Source: CAD feature listing. Evaluate the final solid. Frame: model axes, mm. A direction names the side the tool comes from. Round coordinates to 2 decimals unless told otherwise and drop trailing zeros. Order: outer loops, then holes, each group sorted by start corner. A loop starts at its lowest first (then second) coordinate and runs counter-clockwise, first axis right, second up. Notation, with made-up numbers: (66.5, -27) - (108.5, -27) arc R27 ccw to (108.5, 5) - close; hole circle Ø5 at (72, -30.75). An arc over 180 degrees is marked (long way). Put each result on its own line as item: value. Start each with the question number.
1) Contact query for a flat-ended pin moving along its axis: P1, Ø10.5, axis at x = 305, z = -50, coming from the -Y side. Output: stop coordinate, or through.
2) Section B-B on y = 7.25. State how many separate pieces and enclosed holes the cut face has, then the cut area to 3 significant figures.
3) Access query for faces 5 (the face through (320, 10, 1)), 6 (the face through (-150, 10, 220)), 7 (the face through (-320, 10, -1)). Directions: +Z, -Z, +X, -X, +Y, -Y. A direction counts if a zero-diameter tool reaches every point of the face in a straight line with its end or side. Return the directions, or none.
4) Section A-A on x = 7. Output: boundary loops of the cut face in (y, z).
5) Mould query, pull axis Z, two halves, no side actions, for faces 1 (the face through (375, 10, 164)), 2 (the face through (-2, 10, -210)), 3 (the face through (-2, 10, 230)), 4 (the face through (5, 10, -250)). Classes: +Z half, -Z half, draft (parallel to the pull), parting line (faces both ways), or undercut.
6) Line query: probe 1 along Z at (x, y) = (-360, 14.75); probe 2 along Z at (x, y) = (-89, 15.75); probe 3 along X at (y, z) = (4.5, 50). Output: solid intervals per line, ascending. Write a range as [from, to].
```python
from build123d import *

# Parameters (mm, degrees)
SKETCH1_W                  = 300
SKETCH1_H                  = 20
BOSS_EXTRUDE1_DEPTH        = 20
F_13_0_13_DIAMETER_HOLE1_D = 13


with BuildPart() as part:
    # Sketch1 → Boss-Extrude1 (new body)
    with BuildSketch(Plane(origin=(0, 0, 0), x_dir=(1, 0, 0), z_dir=(0, 1, 0))):
        Polygon((-375, -250), (375, -250), (375, -75), (320, -75), (320, 75), (375, 75), (375, 250), (-375, 250), (-375, 75), (-320, 75), (-320, -75), (-375, -75), align=None)
        with Locations((0, -220)):
            Rectangle(SKETCH1_W, SKETCH1_H, mode=Mode.SUBTRACT)
        with Locations((0, -110)):
            Rectangle(SKETCH1_W, SKETCH1_H, mode=Mode.SUBTRACT)
        with Locations((0, 110)):
            Rectangle(SKETCH1_W, SKETCH1_H, mode=Mode.SUBTRACT)
        with Locations((0, 220)):
            Rectangle(SKETCH1_W, SKETCH1_H, mode=Mode.SUBTRACT)
    extrude(amount=BOSS_EXTRUDE1_DEPTH)

    # Ø13.0 (13) Diameter Hole1 (through all)
    with Locations(Plane(origin=(0, 20, 0), x_dir=(1, 0, 0), z_dir=(0, 1, 0))):
        with Locations((-360, 129), (-305, 50), (-240, 0), (-300, 129), (-300, 185), (-360, 185), (-360, -129), (-360, -185), (-300, -129), (-300, -185), (-305, -50), (360, -129), (300, -129), (360, -185), (360, 129), (360, 185), (300, 129), (305, -50), (300, -185), (300, 185), (240, 0), (305, 50)):
            Hole(F_13_0_13_DIAMETER_HOLE1_D / 2)


solid = part.part
```
Answer sheet:
1. P1: through
2. separate pieces: 1
2. enclosed holes: 26
2. area: 332,000 mm^2
3. face 5: +X, +Y, -Y
3. face 6: +Y, -Y
3. face 7: -X, +Y, -Y
4. outline: (0, -250) - (20, -250) - (20, -230) - (0, -230) - close; (0, -210) - (20, -210) - (20, -120) - (0, -120) - close; (0, -100) - (20, -100) - (20, 100) - (0, 100) - close; (0, 120) - (20, 120) - (20, 210) - (0, 210) - close; (0, 230) - (20, 230) - (20, 250) - (0, 250) - close
5. face 1: draft
5. face 2: undercut
5. face 3: undercut
5. face 4: -Z half
6. probe 1: [-250, -191.5], [-178.5, -135.5], [-122.5, -75], [75, 122.5], [135.5, 178.5], [191.5, 250]
6. probe 2: [-250, -230], [-210, -120], [-100, 100], [120, 210], [230, 250]
6. probe 3: [-320, -311.5], [-298.5, 298.5], [311.5, 320]
